Geometry check sheet. Reference: the model listing, model coordinates, mm. A direction names the side the tool comes from. Coordinates: 2 decimals unless noted, no trailing zeros. Write each loop counter-clockwise with the first axis right and the second up, starting at its lowest first coordinate (ties: lowest second). Pieces come first, ordered by that corner, then holes. Notation, with made-up numbers: M 13,55 L 72,55 A22 ccw 72,78 Z; hole C 38.5,58 d1. An arc over 180 degrees is marked long. Write each question's results on one line, items separated by ' | '.
```python
from build123d import *

# Parameters (mm, degrees)
BASEHEAD_DEPTH = 6.58
SKETCH3_R      = 5
BASEBODY_DEPTH = 100
CHAMFER1_SIZE  = 0.812


with BuildPart() as part:
    # Sketch-BaseHead → BaseHead (new body)
    with BuildSketch(Plane(origin=(0, 0, 0), x_dir=(0, 0, -1), z_dir=(1, 0, 0))):
        Polygon((9.081719734, 0), (4.540859867, 7.865), (-4.540859867, 7.865), (-9.081719734, 0), (-4.540859867, -7.865), (4.540859867, -7.865), align=None)
    extrude(amount=BASEHEAD_DEPTH)

    # Sketch4 → HeadChamfer (revolve, cut)
    with BuildSketch(Plane(origin=(-0.264637255, 0, 5.916896391), x_dir=(0, 0, -1), z_dir=(0, 1, 0))):
        Polygon((14.998616125, -0.264637255), (13.781896391, -0.264637255), (14.998616125, -0.707487022), align=None)
    revolve(axis=Axis((-4.001564945, 0, 0), (1, 0, 0)), mode=Mode.SUBTRACT)

    # Sketch1 → Revolve1 (revolve)
    with BuildSketch(Plane.XY, mode=Mode.PRIVATE) as revolve1_sk:
        Polygon((6.58, 0), (7.08, 0), (7.08, -7.315), (6.58, -7.865), align=None)
    revolve(revolve1_sk.sketch.rotate(Axis((-4.001564945, 0, 0), (1, 0, 0)), 270), axis=Axis((-4.001564945, 0, 0), (1, 0, 0)))

    # Sketch3 → BaseBody (add)
    with BuildSketch(Plane(origin=(7.08, 0, 0), x_dir=(0, 0, -1), z_dir=(1, 0, 0))):
        Circle(SKETCH3_R)
    extrude(amount=BASEBODY_DEPTH)

    # Chamfer1
    chamfer1_edges = [part.edges().sort_by_distance(p)[0] for p in [
        (107.08, 0, 5),
    ]]
    chamfer(chamfer1_edges, length=CHAMFER1_SIZE)


solid = part.part
```
Q1. Scan lines: probe 1 along X at (y, z) = (-6.5, -2); probe 2 along X at (y, z) = (-7, 3); probe 3 along Z at (x, y) = (23.5, 0.25). Record each from-to range of solid material in increasing order.
Geometry check:
probe 1: x = 0 to 7.08 | probe 2: x = 0 to 6.81 | probe 3: z = -4.99 to 4.99
Q2. Sectioned sample at A-A on x = 31.5. Record the cut outline in (y, z).
Geometry check:
outline: C 0,0 d10
Q3. Access from +Z, -Z, +X, -X, +Y, -Y to the whole of each face (thin tool, end or side, straight path). Record for faces 1 (the flat face through (7.08, 2, -5)), 2 (the flat face through (6.58, 7, 4)), 3 (the flat face through (6.58, -7, 4)).
Geometry check:
face 1: +X | face 2: +Z, +X, +Y | face 3: +Z, +X, -Y
Q4. Depth check by flat-ended pin: P1, Ø3, axis at y = -6.5, z = -2.5, coming from the +X side; P2, Ø2, axis at x = 95, z = 2.5, coming from the +Y side; P3, Ø6, axis at x = 64.5, z = 6, coming from the -Y side. Enter the tip coordinate at first touch or a pass-through.
Geometry check:
P1: stops at x = 7.08 | P2: stops at y = 4.77 | P3: stops at y = -4
